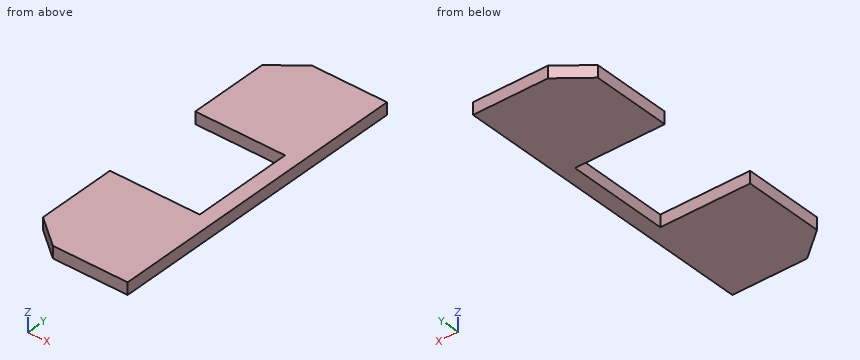
```python
from build123d import *

# Parameters (mm, degrees)
SKETCH1_W      = 15
SKETCH1_H      = 310
EXTRUDE1_DEPTH = 6
EXTRUDE3_DEPTH = 6


with BuildPart() as part:
    # Sketch1 → Extrude1 (new, symmetric)
    with BuildSketch(Plane.XY):
        Rectangle(SKETCH1_W, SKETCH1_H)
    extrude(amount=EXTRUDE1_DEPTH, both=True)

    # Sketch3 → Extrude3 (add, symmetric)
    with BuildSketch(Plane.XY):
        Polygon((-7.5, 155), (-67.5, 155), (-97.5, 131), (-97.5, 51), (-7.5, 51), align=None)
        Polygon((-7.5, -51), (-7.5, -155), (-67.5, -155), (-97.5, -131), (-97.5, -51), align=None)
    extrude(amount=EXTRUDE3_DEPTH, both=True)


solid = part.part
```
Model file for the job. Use its own axes, mm. Coordinates: 2 decimals unless noted, no trailing zeros. Order: outer loops, then holes, each group sorted by start corner. A loop starts at its lowest first (then second) coordinate and runs counter-clockwise, first axis right, second up. Notation, with made-up numbers: M 1,56 L 7,56 A14 cw 7,61 Z; hole C -33,72 d1. An arc over 180 degrees is marked long. Answer as CSV lines item,"result".
(1) Wall check: line 1 along Y through (x, z) = (-40, -3.75); line 2 along X through (y, z) = (0, 5); line 3 along Y through (x, z) = (-82, 4.5). Give the ranges that are in metal, low to high.
Geometry says:
line 1,"y = -155 to -51, 51 to 155"
line 2,"x = -7.5 to 7.5"
line 3,"y = -143.4 to -51, 51 to 143.4"
(2) Band-saw the part on B-B, the plane z = -0.5. List the corners of the cut face in (x, y), then the cut area to 4 significant figures.
Geometry says:
outline,"M -97.5,-131 L -67.5,-155 L 7.5,-155 L 7.5,155 L -67.5,155 L -97.5,131 L -97.5,51 L -7.5,51 L -7.5,-51 L -97.5,-51 Z"
area,"22,650 mm2"
(3) Flat gauge pin, fed straight in: pin 1 (2 mm diameter, centred on y = -40, z = -0.5, fed in from -X). Where does the tip first touch, or does it go through?
Geometry says:
pin 1,"stops at x = -7.5"
(4) Band-saw the part on D-D, the plane y = -30. List the corners of the cut face in (x, z), then the cut area to 3 significant figures.
Geometry says:
outline,"M -7.5,-6 L 7.5,-6 L 7.5,6 L -7.5,6 Z"
area,"180 mm2"
(5) Band-saw the part on C-C, the plane x = -47.5. List the corners of the cut face in (y, z), then the cut area to 3 significant figures.
Geometry says:
outline,"M -155,-6 L -51,-6 L -51,6 L -155,6 Z; M 51,-6 L 155,-6 L 155,6 L 51,6 Z"
area,"2,500 mm2"
(6) Band-saw the part on A-A, the plane x = -78.5. List the corners of the cut face in (y, z).
Geometry says:
outline,"M -146.2,-6 L -51,-6 L -51,6 L -146.2,6 Z; M 51,-6 L 146.2,-6 L 146.2,6 L 51,6 Z"
